from build123d import *

# Parameters (mm, degrees)
SKETCH1_R           = 50
BOSS_EXTRUDE1_DEPTH = 10


with BuildPart() as part:
    # Sketch1 → Boss-Extrude1 (new body)
    with BuildSketch(Plane.XY):
        with BuildLine():
            Line((12, 0), (120, 0))
            ThreePointArc((120, 0), (170, 50), (220, 0))
            Line((220, 0), (328, 0))
            Line((328, 0), (340, 12))
            Line((340, 12), (340, 338))
            Line((340, 338), (328, 350))
            Line((328, 350), (220, 350))
            ThreePointArc((220, 350), (170, 300), (120, 350))
            Line((120, 350), (12, 350))
            Line((12, 350), (0, 338))
            Line((0, 338), (0, 12))
            Line((0, 12), (12, 0))
        make_face()
        with Locations((170, 175)):
            Circle(SKETCH1_R, mode=Mode.SUBTRACT)
        with Locations((87.5, 279)):
            Circle(SKETCH1_R, mode=Mode.SUBTRACT)
        with Locations((262.5, 279)):
            Circle(SKETCH1_R, mode=Mode.SUBTRACT)
        with Locations(Location((87.5, 71, 0), (0, 0, 180))):
            Circle(SKETCH1_R, mode=Mode.SUBTRACT)
        with Locations(Location((262.5, 71, 0), (0, 0, 180))):
            Circle(SKETCH1_R, mode=Mode.SUBTRACT)
    extrude(amount=BOSS_EXTRUDE1_DEPTH)


solid = part.part
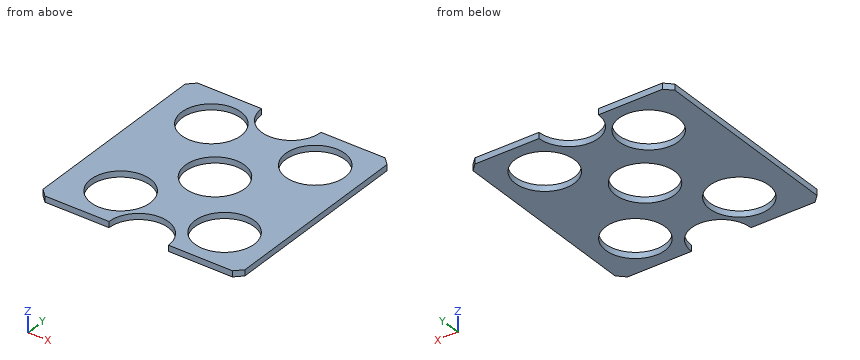
Can you work these out from the model? Positions are in its coordinate system, mm. Coordinates: 2 decimals unless noted, no trailing zeros. Write each loop counter-clockwise with the first axis right and the second up, starting at its lowest first coordinate (ties: lowest second). Pieces come first, ordered by that corner, then holes.
Q1. For P1, Ø1.5, axis at y = 136, z = 4.5, coming from the -X side; P2, Ø1, axis at x = 129, z = 7, coming from the +Y side, each with a flat end and sliding along its axis, tell me the tip position at first contact or that it passes through.
Results found:
P1: stops at x = 0
P2: stops at y = 322.11
Q2. Imagine slicing it at C-C, the plane z = 4.25. List the corners of the cut face in (x, y) for me.
Results found:
outline: (0, 12) - (12, 0) - (120, 0) arc R50 cw to (220, 0) - (328, 0) - (340, 12) - (340, 338) - (328, 350) - (220, 350) arc R50 cw to (120, 350) - (12, 350) - (0, 338) - close; hole circle Ø100 at (87.5, 71); hole circle Ø100 at (87.5, 279); hole circle Ø100 at (170, 175); hole circle Ø100 at (262.5, 71); hole circle Ø100 at (262.5, 279)
Q3. Imagine slicing it at B-B, the plane y = 279. List the corners of the cut face in (x, z) for me.
Results found:
outline: (0, 0) - (37.5, 0) - (37.5, 10) - (0, 10) - close; (137.5, 0) - (212.5, 0) - (212.5, 10) - (137.5, 10) - close; (312.5, 0) - (340, 0) - (340, 10) - (312.5, 10) - close
Q4. Please list where these lines run through material, in increasing order: L1, parallel to X at y = 71, z = 7; L2, parallel to Y at x = 87.5, z = 3.25; L3, parallel to Y at x = 243.5, z = 7.25.
Results found:
L1: x = 0 to 37.5, 137.5 to 212.5, 312.5 to 340
L2: y = 0 to 21, 121 to 229, 329 to 350
L3: y = 0 to 24.75, 117.25 to 232.75, 325.25 to 350
Q5. Imagine slicing it at A-A, the plane x = 87.5. List the corners of the cut face in (y, z) for me.
Results found:
outline: (0, 0) - (21, 0) - (21, 10) - (0, 10) - close; (121, 0) - (229, 0) - (229, 10) - (121, 10) - close; (329, 0) - (350, 0) - (350, 10) - (329, 10) - close
Q6. Imagine slicing it at D-D, the plane x = 170. List the corners of the cut face in (y, z) for me.
Results found:
outline: (50, 0) - (125, 0) - (125, 10) - (50, 10) - close; (225, 0) - (300, 0) - (300, 10) - (225, 10) - close
